from build123d import *
from OCP.BRepFilletAPI import BRepFilletAPI_MakeFillet

# Parameters (mm, degrees)
L_BRACKET_BODY_DEPTH             = 40
ARC_SLOT_R50_30DEG_REACH         = 168.433
CORNER_ROUNDS_R1                 = 20
CORNER_ROUNDS_R2                 = 15
COUNTERBORED_HOLE_12_D           = 12
COUNTERBORED_HOLE_12_DEPTH       = 100
COUNTERBORED_HOLE_12_CBORE_D     = 25
COUNTERBORED_HOLE_12_CBORE_DEPTH = 5
UPRIGHT_HOLES_2X_REACH           = 161.531
UPRIGHT_HOLES_SKETCH_R           = 7.5


with BuildPart() as part:
    # L Profile Sketch → L Bracket Body (new, symmetric)
    with BuildSketch(Plane.XY):
        Polygon((0, 0), (0, 75), (15, 75), (15, 15), (150, 15), (150, 0), align=None)
    extrude(amount=L_BRACKET_BODY_DEPTH, both=True)

    # Arc Slot Sketch → Arc Slot R50 30deg (cut, up to next)
    with BuildSketch(Plane(origin=(0, 15, 0), x_dir=(1, 0, 0), z_dir=(0, 1, 0)), mode=Mode.PRIVATE) as arc_slot_r50_30deg_sk1:
        with BuildLine():
            Line((138.442887702, -40), (150, -40))
            Line((150, -40), (150, 0))
            ThreePointArc((150, 0), (147.052815967, -20.818062138), (138.442887702, -40))
        make_face()
    arc_slot_r50_30deg_tool1 = extrude(arc_slot_r50_30deg_sk1.sketch, amount=-ARC_SLOT_R50_30DEG_REACH, mode=Mode.PRIVATE) & part.part
    # Arc Slot Sketch → Arc Slot R50 30deg (cut, up to next)
    with BuildSketch(Plane(origin=(0, 15, 0), x_dir=(1, 0, 0), z_dir=(0, 1, 0)), mode=Mode.PRIVATE) as arc_slot_r50_30deg_sk2:
        with BuildLine():
            ThreePointArc((138.442887702, 40), (147.052815967, 20.818062138), (150, 0))
            Line((150, 0), (150, 40))
            Line((150, 40), (138.442887702, 40))
        make_face()
    arc_slot_r50_30deg_tool2 = extrude(arc_slot_r50_30deg_sk2.sketch, amount=-ARC_SLOT_R50_30DEG_REACH, mode=Mode.PRIVATE) & part.part
    # Arc Slot Sketch → Arc Slot R50 30deg (cut, up to next)
    with BuildSketch(Plane(origin=(0, 15, 0), x_dir=(1, 0, 0), z_dir=(0, 1, 0)), mode=Mode.PRIVATE) as arc_slot_r50_30deg_sk3:
        with BuildLine():
            ThreePointArc((125.229473419, -29), (133, 0), (125.229473419, 29))
            ThreePointArc((125.229473419, 29), (114.301270189, 31.92820323), (111.373066959, 21))
            ThreePointArc((111.373066959, 21), (117, 0), (111.373066959, -21))
            ThreePointArc((111.373066959, -21), (114.301270189, -31.92820323), (125.229473419, -29))
        make_face()
    arc_slot_r50_30deg_tool3 = extrude(arc_slot_r50_30deg_sk3.sketch, amount=-ARC_SLOT_R50_30DEG_REACH, mode=Mode.PRIVATE) & part.part
    add(arc_slot_r50_30deg_tool1.solids().sort_by_distance((146.584015, 15, 30.160634))[0], mode=Mode.SUBTRACT)
    add(arc_slot_r50_30deg_tool2.solids().sort_by_distance((146.584015, 15, -30.160634))[0], mode=Mode.SUBTRACT)
    add(arc_slot_r50_30deg_tool3.solids().sort_by_distance((121.886119, 15, 0))[0], mode=Mode.SUBTRACT)

    # Corner Rounds: one fillet with a radius per group of edges: ONE call of the kernel's fillet builder (fillet() takes one radius for all edges)
    corner_rounds_edges_1 = [part.edges().sort_by_distance(p)[0] for p in [
        (138.442887702, 7.5, 40),
        (138.442887702, 7.5, -40),
    ]]
    corner_rounds_edges_2 = [part.edges().sort_by_distance(p)[0] for p in [
        (7.5, 75, 40),
        (7.5, 75, -40),
    ]]
    corner_rounds = BRepFilletAPI_MakeFillet(part.part.solid().wrapped)
    for e in corner_rounds_edges_1:
        corner_rounds.Add(CORNER_ROUNDS_R1, e.wrapped)
    for e in corner_rounds_edges_2:
        corner_rounds.Add(CORNER_ROUNDS_R2, e.wrapped)
    add(Compound.cast(corner_rounds.Shape()), mode=Mode.REPLACE)

    # Counterbored Hole _12
    with Locations(Plane(origin=(0, 15, 0), x_dir=(1, 0, 0), z_dir=(0, 1, 0))):
        with Locations((75, 0)):
            CounterBoreHole(COUNTERBORED_HOLE_12_D / 2, COUNTERBORED_HOLE_12_CBORE_D / 2, COUNTERBORED_HOLE_12_CBORE_DEPTH, depth=COUNTERBORED_HOLE_12_DEPTH)

    # Upright Holes Sketch → Upright Holes 2x (cut, up to next)
    with BuildSketch(Plane(origin=(15, 0, 0), x_dir=(0, 0, -1), z_dir=(1, 0, 0)), mode=Mode.PRIVATE) as upright_holes_2x_sk1:
        with Locations(Location((-25, 60, 0), (0, 0, 90))):
            Circle(UPRIGHT_HOLES_SKETCH_R)
    upright_holes_2x_tool1 = extrude(upright_holes_2x_sk1.sketch, amount=-UPRIGHT_HOLES_2X_REACH, mode=Mode.PRIVATE) & part.part
    # Upright Holes Sketch → Upright Holes 2x (cut, up to next)
    with BuildSketch(Plane(origin=(15, 0, 0), x_dir=(0, 0, -1), z_dir=(1, 0, 0)), mode=Mode.PRIVATE) as upright_holes_2x_sk2:
        with Locations(Location((25, 60, 0), (0, 0, 90))):
            Circle(UPRIGHT_HOLES_SKETCH_R)
    upright_holes_2x_tool2 = extrude(upright_holes_2x_sk2.sketch, amount=-UPRIGHT_HOLES_2X_REACH, mode=Mode.PRIVATE) & part.part
    add(upright_holes_2x_tool1.solids().sort_by_distance((15, 60, 25))[0], mode=Mode.SUBTRACT)
    add(upright_holes_2x_tool2.solids().sort_by_distance((15, 60, -25))[0], mode=Mode.SUBTRACT)


solid = part.part
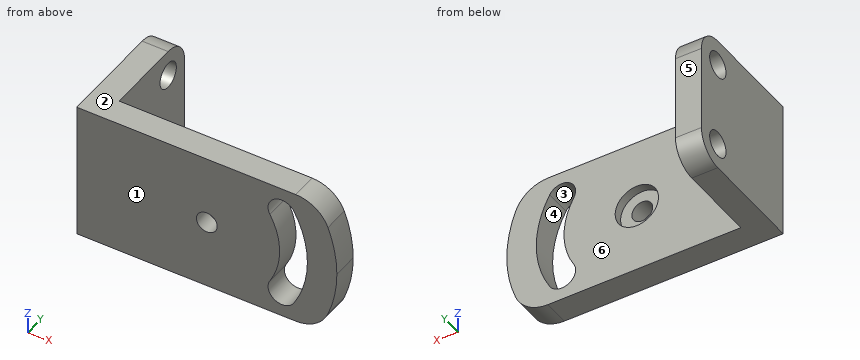
Here's how the part is built. I have some questions about the finished solid (model axes, mm). Face numbers are marked on the shaded views. A direction names the side the tool comes from. Coordinates: 2 decimals unless noted, no trailing zeros. Order: outer loops, then holes, each group sorted by start corner. A loop starts at its lowest first (then second) coordinate and runs counter-clockwise, first axis right, second up. Notation, with made-up numbers: M 3,76 L 48,76 A6 cw 48,83 Z; hole C 7.25,-22.5 d8. An arc over 180 degrees is marked long. Answer as CSV lines item,"result". Start each with the question number.
1. I want a section at D-D, the plane z = -35. Write out the boundary of the cut face in (x, y).
2. I need wall thicknesses on line 1 (Z direction, x = 6, y = 60); line 2 (Z direction, x = 75, y = 12.7); line 3 (X direction, y = 65, z = -35). Which ranges of each line are inside material? Lowest first, please. Write a range as [from, to].
3. I want a section at C-C, the plane x = 40. Write out the boundary of the cut face in (y, z), and give its area (3 significant figures).
4. On a 3-axis mill with a long thin cutter (end or side, diameter ignored), from which of +Z, -Z, +X, -X, +Y, -Y can I reach the whole of each face in a straight line? I mean the marked faces 4, 5 and 6. Say none if no direction works.
5. I want a section at A-A, the plane x = 75. Write out the boundary of the cut face in (y, z).
6. We'd pull the mould along Z, two halves only. Please class the marked faces 1, 2 and 3: released by +Z, released by -Z, zero draft, split by the parting line, or undercut.
7. I want a section at B-B, the plane y = 55.5. Write out the boundary of the cut face in (x, z), and give its area (3 significant figures).
8. For pin 1 (12 mm diameter, centred on y = 60, z = 25, fed in from +X); pin 2 (12 mm diameter, centred on x = 39.5, z = 10, fed in from +Y); pin 3 (2 mm diameter, centred on y = 64, z = -16, fed in from +X); pin 4 (1.5 mm diameter, centred on y = 8, z = -19, fed in from +X), each with a flat end and sliding along its axis, tell me the tip position at first contact or that it passes through.
Recorded:
1,outline,"M 0,0 L 139.46,0 L 139.46,15 L 15,15 L 15,71.18 L 0,71.18 Z"
2,line 1,"z = [-40, -32.5], [-17.5, 17.5], [32.5, 40]"
2,line 2,"z = [-40, -12.5], [12.5, 40]"
2,line 3,"x = [0, 15]"
3,outline,"M 0,-40 L 15,-40 L 15,40 L 0,40 Z"
3,area,"1,200 mm2"
4,face 4,"+Y, -Y"
4,face 5,"+Z, -Z, +X, -X, +Y"
4,face 6,"+Z, -Z, +X, +Y"
5,outline,"M 0,-40 L 15,-40 L 15,-12.5 L 10,-12.5 L 10,-6 L 0,-6 Z; M 0,6 L 10,6 L 10,12.5 L 15,12.5 L 15,40 L 0,40 Z"
6,face 1,"zero draft"
6,face 2,"released by +Z"
6,face 3,"undercut"
7,outline,"M 0,-40 L 15,-40 L 15,-31 L 0,-31 Z; M 0,-19 L 15,-19 L 15,19 L 0,19 Z; M 0,31 L 15,31 L 15,40 L 0,40 Z"
7,area,"840 mm2"
8,pin 1,"passes through"
8,pin 2,"stops at y = 15"
8,pin 3,"stops at x = 15"
8,pin 4,"stops at x = 147.75"
